Can you work these out from the model? Positions are in its coordinate system, mm. Round coordinates to 2 decimals unless told otherwise and drop trailing zeros. Loops run counter-clockwise (first coordinate to the right, second up) from the corner with the lowest first, then second, coordinate; pieces in that order, holes last.
(1) Will this pin go through, and if not, where does the flat tip stop? pin 1 Ø4.5 at (x, y) = (146.5, -7.5) entering from -Z.
(2) I want a section at A-A on x = 145. Write out the boundary of the cut face in (y, z).
(3) I want a section at C-C on y = -124. Write out the boundary of the cut face in (x, z), plus the area to 4 significant figures.
(4) If I drill on line 1 along Y through (x, z) = (102.5, 3); line 2 along X through (y, z) = (-50, 0); line 3 along X through (y, z) = (-41.5, 6), over which ranges is the centre line in solid material (lowest first)?
(5) I want a section at B-B on z = -3.25. Give the number of separate pieces and of enclosed holes in the cut face, plus the area to 3 significant figures.
(6) I want a section at D-D on x = 48.5. Write out the boundary of the cut face in (y, z).
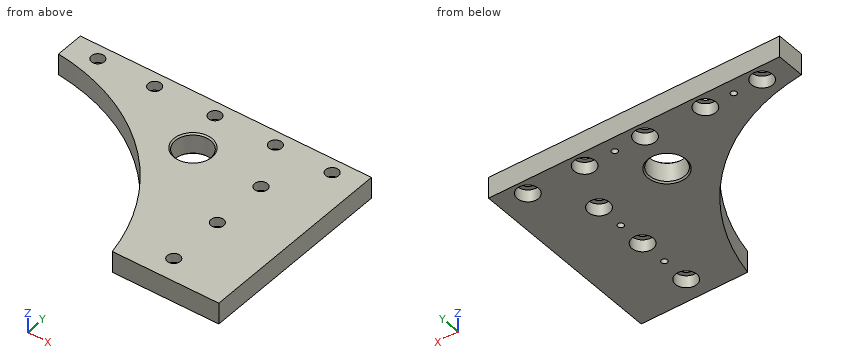
from build123d import *

# Parameters (mm, degrees)
EXTRUDE_1_DEPTH              = 7.5
HOLE_WIZARD_M8_2_D           = 9
HOLE_WIZARD_M8_2_CBORE_D     = 15
HOLE_WIZARD_M8_2_CBORE_DEPTH = 8.6
HOLE_WIZARD_M5_1_D           = 4.2
HOLE_WIZARD_M5_1_DEPTH       = 12.4
HOLE_WIZARD_M5_1_TIP         = 1.2618073
SKETCH_11_R                  = 150
CUT_EXTRUDE_4_DEPTH          = 249.696602309
SKETCH_12_R                  = 12.5
CUT_EXTRUDE_5_DEPTH          = 249.696602309
CHAMFER_1_SIZE               = 1


with BuildPart() as part:
    # 草图1 → 凸台-拉伸1 (new, symmetric)
    with BuildSketch(Plane.XY):
        Polygon((0, 0), (205, 0), (205, -140), (130, -140), (0, -20), align=None)
    extrude(amount=EXTRUDE_1_DEPTH, both=True)

    # M8 六角凹头螺钉的柱形沉头孔2 (through all)
    with Locations(Plane(origin=(0, 0, -7.5), x_dir=(1, 0, 0), z_dir=(0, 0, -1))):
        with Locations((20, 10), (60, 10), (102.5, 10), (145, 10), (161, 44), (161, 84), (161, 124), (185, 10)):
            CounterBoreHole(HOLE_WIZARD_M8_2_D / 2, HOLE_WIZARD_M8_2_CBORE_D / 2, HOLE_WIZARD_M8_2_CBORE_DEPTH)

    # M5 螺纹孔1
    with Locations(Plane(origin=(0, 0, -7.5), x_dir=(1, 0, 0), z_dir=(0, 0, -1))):
        with Locations((40, 10), (123.75, 10), (161, 64), (161, 104)):
            Hole(HOLE_WIZARD_M5_1_D / 2, depth=HOLE_WIZARD_M5_1_DEPTH)
            with Locations((0, 0, -(HOLE_WIZARD_M5_1_DEPTH + HOLE_WIZARD_M5_1_TIP / 2))):  # 118° drill point
                Cone(0, HOLE_WIZARD_M5_1_D / 2, HOLE_WIZARD_M5_1_TIP, mode=Mode.SUBTRACT)

    # 草图11 → 切除-拉伸4 (cut, through all)
    with BuildSketch(Plane.XY.offset(7.5)):
        with Locations((-17.167132722, -169.014393782)):
            Circle(SKETCH_11_R)
    extrude(amount=-CUT_EXTRUDE_4_DEPTH, mode=Mode.SUBTRACT)

    # 草图12 → 切除-拉伸5 (cut, through all)
    with BuildSketch(Plane(origin=(0, 0, -7.5), x_dir=(-1, 0, 0), z_dir=(0, 0, -1))):
        with Locations((-110, -40)):
            Circle(SKETCH_12_R)
    extrude(amount=-CUT_EXTRUDE_5_DEPTH, mode=Mode.SUBTRACT)

    # 倒角1
    chamfer_1_edges = [part.edges().sort_by_distance(p)[0] for p in [
        (122.5, -40, 7.5),
        (122.5, -40, -7.5),
    ]]
    chamfer(chamfer_1_edges, length=CHAMFER_1_SIZE)


solid = part.part
Filled sheet:
1. pin 1: stops at z = 1.1
2. outline: (-140, -7.5) - (-17.5, -7.5) - (-17.5, 1.1) - (-14.5, 1.1) - (-14.5, 7.5) - (-140, 7.5) - close; (-5.5, 1.1) - (-2.5, 1.1) - (-2.5, -7.5) - (0, -7.5) - (0, 7.5) - (-5.5, 7.5) - close
3. outline: (125.92, -7.5) - (153.5, -7.5) - (153.5, 1.1) - (156.5, 1.1) - (156.5, 7.5) - (125.92, 7.5) - close; (165.5, 1.1) - (168.5, 1.1) - (168.5, -7.5) - (205, -7.5) - (205, 7.5) - (165.5, 7.5) - close
3. area: 1,000 mm2
4. line 1: y = -78.57 to -50, -30 to -14.5, -5.5 to 0
4. line 2: x = 74.13 to 102.5, 117.5 to 156.5, 165.5 to 205
4. line 3: x = 61.83 to 97.59, 122.41 to 157.26, 164.74 to 205
5. separate pieces: 1
5. enclosed holes: 13
5. area: 15,500 mm2
6. outline: (-34.15, -7.5) - (0, -7.5) - (0, 7.5) - (-34.15, 7.5) - close
